from build123d import *

# Parameters (mm, degrees)
SKETCH1_R           = 230
SKETCH1_R_2         = 191
BOSS_EXTRUDE1_DEPTH = 0.5
SKETCH2_R           = 9
CUT_EXTRUDE2_DEPTH  = 0.5
CIRPATTERN1_COUNT   = 6


with BuildPart() as part:
    # Sketch1 → Boss-Extrude1 (new, symmetric)
    with BuildSketch(Plane(origin=(0, 0, 0), x_dir=(1, 0, 0), z_dir=(0, 1, 0))):
        with Locations(Location((0, 0, 0), (0, 0, 270))):
            Circle(SKETCH1_R)
        with Locations(Location((0, 0, 0), (0, 0, 270))):
            Circle(SKETCH1_R_2, mode=Mode.SUBTRACT)
    extrude(amount=BOSS_EXTRUDE1_DEPTH, both=True)

    # Sketch2 → Cut-Extrude2 (cut, symmetric)
    with BuildSketch(Plane(origin=(0, 0, 0), x_dir=(1, 0, 0), z_dir=(0, 1, 0))):
        with Locations(Location((-210, 0, 0), (0, 0, 270))):
            Circle(SKETCH2_R)
    cut_extrude2 = extrude(amount=CUT_EXTRUDE2_DEPTH, both=True, mode=Mode.SUBTRACT)

    # CirPattern1: Cut-Extrude2 ×6 about axis
    cirpattern1_axis = Axis((0, 0, 0), (0, 1, 0))
    for i in range(1, CIRPATTERN1_COUNT):
        add(cut_extrude2.rotate(cirpattern1_axis, i * 360 / CIRPATTERN1_COUNT), mode=Mode.SUBTRACT)


solid = part.part
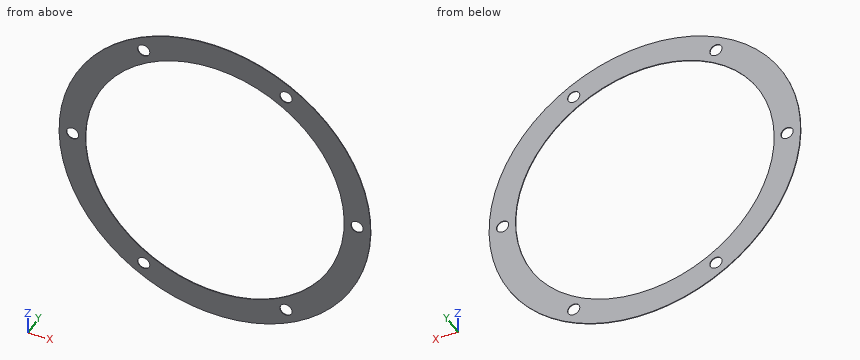
Here's how the part is built. I have some questions about the finished solid (model axes, mm). Coordinates: 2 decimals unless noted, no trailing zeros. Order: outer loops, then holes, each group sorted by start corner. A loop starts at its lowest first (then second) coordinate and runs counter-clockwise, first axis right, second up. Notation, with made-up numbers: M 41.5,64.5 L 51.5,64.5 A16 ccw 51.5,71.5 Z; hole C 79.25,80.5 d8. An arc over 180 degrees is marked long. Answer as CSV lines item,"result".
Item 1: Imagine slicing it at D-D on x = -105. Write out the boundary of the cut face in (y, z), plus the area to 3 significant figures.
Results found:
outline,"M -0.5,-204.63 L 0.5,-204.63 L 0.5,-190.87 L -0.5,-190.87 Z; M -0.5,-172.87 L 0.5,-172.87 L 0.5,-159.55 L -0.5,-159.55 Z; M -0.5,159.55 L 0.5,159.55 L 0.5,172.87 L -0.5,172.87 Z; M -0.5,190.87 L 0.5,190.87 L 0.5,204.63 L -0.5,204.63 Z"
area,"54.2 mm2"
Item 2: For pin 1 (14.5 mm diameter, centred on x = 105, z = -181.87, fed in from -Y), with a flat end and sliding along its axis, tell me the tip position at first contact or that it passes through.
Results found:
pin 1,"through"
Item 3: Imagine slicing it at A-A on x = 0. Write out the boundary of the cut face in (y, z).
Results found:
outline,"M -0.5,-230 L 0.5,-230 L 0.5,-191 L -0.5,-191 Z; M -0.5,191 L 0.5,191 L 0.5,230 L -0.5,230 Z"
Item 4: Imagine slicing it at C-C on z = 66.5. Write out the boundary of the cut face in (x, y).
Results found:
outline,"M -220.18,-0.5 L -179.05,-0.5 L -179.05,0.5 L -220.18,0.5 Z; M 179.05,-0.5 L 220.18,-0.5 L 220.18,0.5 L 179.05,0.5 Z"
Item 5: Imagine slicing it at B-B on z = 0. Write out the boundary of the cut face in (x, y), plus the area to 3 significant figures.
Results found:
outline,"M -230,-0.5 L -219,-0.5 L -219,0.5 L -230,0.5 Z; M -201,-0.5 L -191,-0.5 L -191,0.5 L -201,0.5 Z; M 191,-0.5 L 201,-0.5 L 201,0.5 L 191,0.5 Z; M 219,-0.5 L 230,-0.5 L 230,0.5 L 219,0.5 Z"
area,"42.0 mm2"
Item 6: If I drill on line 1 (X direction, y = 0.15, z = 0); line 2 (Z direction, x = -108, y = 0.05); line 3 (Z direction, x = -1, y = 0.3), over which ranges is the centre line in solid material (lowest first)?
Results found:
line 1,"-230 to -219, -201 to -191, 191 to 201, 219 to 230"
line 2,"-203.07 to -190.35, -173.38 to -157.53, 157.53 to 173.38, 190.35 to 203.07"
line 3,"-230 to -191, 191 to 230"
